Build history of the part. All positions in model axes, mm. Face numbers are marked on the shaded views. A direction names the side the tool comes from. Coordinates: 2 decimals unless noted, no trailing zeros. Write each loop counter-clockwise with the first axis right and the second up, starting at its lowest first coordinate (ties: lowest second). Pieces come first, ordered by that corner, then holes.
from build123d import *

# Parameters (mm, degrees)
BACK_PLATE_PROFILE_W        = 120
BACK_PLATE_PROFILE_H        = 100
BACK_PLATE_120X100X20_DEPTH = 20
TOP_ARM_PROFILE_W           = 120
TOP_ARM_PROFILE_H           = 20
TOP_ARM_80_DEPTH            = 80
SLOT_1_CUT_DEPTH            = 176.499287748
SLOT_2_CUT_DEPTH            = 176.499287748
SLOT_3_CUT_DEPTH            = 176.499287748
ARM_ROOT_FILLET_R10_R       = 10
ARM_CORNER_ROUND_R20_R      = 20
BACK_PLATE_CUT_30_DEPTH     = 176.499287748
BOSS_A_SKETCH_R             = 8
BOSS_A_SKETCH_R_2           = 6
MOUNTING_BOSS_A_DEPTH       = 10
BOSS_B_SKETCH_R             = 8
BOSS_B_SKETCH_R_2           = 6
MOUNTING_BOSS_B_DEPTH       = 10
BOSS_EDGE_FILLET_R2_R       = 2


with BuildPart() as part:
    # Back Plate Profile → Back Plate 120x100x20 (new body)
    with BuildSketch(Plane.XY):
        with Locations((60, 50)):
            Rectangle(BACK_PLATE_PROFILE_W, BACK_PLATE_PROFILE_H)
    extrude(amount=BACK_PLATE_120X100X20_DEPTH)

    # Top Arm Profile → Top Arm 80 (add)
    with BuildSketch(Plane.XY.offset(20)):
        with Locations((60, 90)):
            Rectangle(TOP_ARM_PROFILE_W, TOP_ARM_PROFILE_H)
    extrude(amount=TOP_ARM_80_DEPTH)

    # Slot 1 Sketch → Slot 1 Cut (cut, through all)
    with BuildSketch(Plane.XZ.offset(-80)):
        with BuildLine():
            Line((20, 86), (100, 86))
            ThreePointArc((100, 86), (106, 80), (100, 74))
            Line((100, 74), (20, 74))
            ThreePointArc((20, 74), (14, 80), (20, 86))
        make_face()
    extrude(amount=-SLOT_1_CUT_DEPTH, mode=Mode.SUBTRACT)

    # Slot 2 Sketch → Slot 2 Cut (cut, through all)
    with BuildSketch(Plane.XZ.offset(-80)):
        with BuildLine():
            Line((20, 66), (100, 66))
            ThreePointArc((100, 66), (106, 60), (100, 54))
            Line((100, 54), (20, 54))
            ThreePointArc((20, 54), (14, 60), (20, 66))
        make_face()
    extrude(amount=-SLOT_2_CUT_DEPTH, mode=Mode.SUBTRACT)

    # Slot 3 Sketch → Slot 3 Cut (cut, through all)
    with BuildSketch(Plane.XZ.offset(-80)):
        with BuildLine():
            Line((20, 46.364855501), (100, 46.364855501))
            ThreePointArc((100, 46.364855501), (106.364855501, 40), (100, 33.635144499))
            Line((100, 33.635144499), (20, 33.635144499))
            ThreePointArc((20, 33.635144499), (13.635144499, 40), (20, 46.364855501))
        make_face()
    extrude(amount=-SLOT_3_CUT_DEPTH, mode=Mode.SUBTRACT)

    # Arm Root Fillet R10
    arm_root_fillet_r10_edges = [part.edges().sort_by_distance(p)[0] for p in [
        (60, 80, 20),
    ]]
    fillet(arm_root_fillet_r10_edges, radius=ARM_ROOT_FILLET_R10_R)

    # Arm Corner Round R20
    arm_corner_round_r20_edges = [part.edges().sort_by_distance(p)[0] for p in [
        (0, 90, 100),
        (120, 90, 100),
    ]]
    fillet(arm_corner_round_r20_edges, radius=ARM_CORNER_ROUND_R20_R)

    # Back Plate Cut Sketch → Back Plate Cut 30 (cut, through all)
    with BuildSketch(Plane.XY.offset(20)):
        with BuildLine():
            Line((45, 35), (45, 0))
            Line((45, 0), (75, 0))
            Line((75, 0), (75, 35))
            ThreePointArc((75, 35), (60, 50), (45, 35))
        make_face()
    extrude(amount=-BACK_PLATE_CUT_30_DEPTH, mode=Mode.SUBTRACT)

    # Boss A Sketch → Mounting Boss A (add)
    with BuildSketch(Plane.XY.offset(20)):
        with Locations((30, 30)):
            Circle(BOSS_A_SKETCH_R)
        with Locations((30, 30)):
            Circle(BOSS_A_SKETCH_R_2, mode=Mode.SUBTRACT)
    extrude(amount=MOUNTING_BOSS_A_DEPTH)

    # Boss B Sketch → Mounting Boss B (add)
    with BuildSketch(Plane.XY.offset(20)):
        with Locations((90, 30)):
            Circle(BOSS_B_SKETCH_R)
        with Locations((90, 30)):
            Circle(BOSS_B_SKETCH_R_2, mode=Mode.SUBTRACT)
    extrude(amount=MOUNTING_BOSS_B_DEPTH)

    # Boss Edge Fillet R2
    boss_edge_fillet_r2_edges = [part.edges().sort_by_distance(p)[0] for p in [
        (22, 30, 20),
        (82, 30, 20),
    ]]
    fillet(boss_edge_fillet_r2_edges, radius=BOSS_EDGE_FILLET_R2_R)


solid = part.part
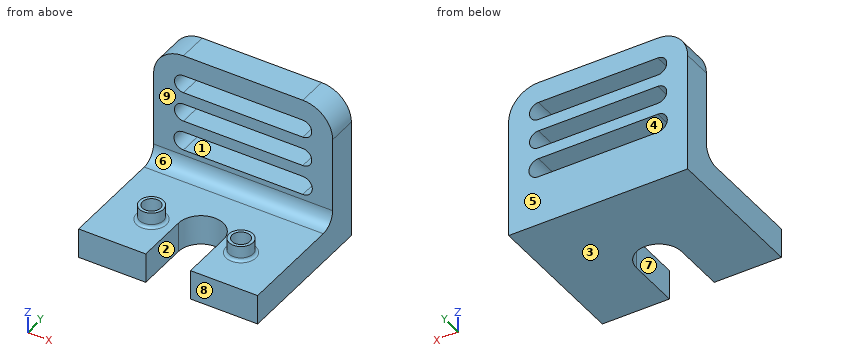
(1) Slice it at B-B, the plane y = 17.5. List the corners of the cut face in (x, z).
(2) Slice it at A-A, the plane x = 30. Give the number of separate pieces and of enclosed holes in the cut face, and give its area (3 significant figures).
(3) Two-plate mould, pull along Z, no slides. Class the marked faces 1, 2, 3 and 4: pulls with the +Z half, pulls with the -Z half, needs draft (parallel to the pull), parting line crosses it, or undercut.
(4) 3-axis set-ups, long thin cutter, end or side, ignore diameter. For the marked faces 5, 6, 7, 8 and 9: which of +Z, -Z, +X, -X, +Y, -Y reach the whole face in a straight line?
(5) Probe L1, parallel to Z at x = 92, y = 93.5; L2, parallel to Y at x = 30, z = 26.25; L3, parallel to Y at x = 90, z = 25.5. List the from-to ranges inside material, lowest first.
(6) Slice it at C-C, the plane z = 60. List the corners of the cut face in (x, y).
(7) Slice it at D-D, the plane z = 12.5. List the corners of the cut face in (x, y).
(8) Flat gauge pins, fed straight in: P1, Ø3.5, axis at x = 92, y = 29, coming from the +Z side; P2, Ø14, axis at x = 90, y = 30, coming from the +Z side; P3, Ø2, axis at x = 106, z = 46.5, coming from the -Y side. Where does each tip first touch, or does it go through?
Results:
1. outline: (0, 0) - (45, 0) - (45, 20) - (0, 20) - close; (75, 0) - (120, 0) - (120, 20) - (75, 20) - close
2. separate pieces: 4
2. enclosed holes: 0
2. area: 2,930 mm2
3. face 1: undercut
3. face 2: needs draft
3. face 3: pulls with the -Z half
3. face 4: undercut
4. face 5: +Z, -Z, +X, -X, +Y
4. face 6: +Z, +X, -X
4. face 7: +Z, -Z, -Y
4. face 8: +Z, -Z, +X, -X, -Y
4. face 9: +Z, +X, -X, -Y
5. L1: z = 0 to 33.64, 46.36 to 54, 66 to 74, 86 to 100
5. L2: y = 22 to 24, 36 to 38, 79.27 to 100
5. L3: y = 22 to 24, 36 to 38, 78.93 to 100
6. outline: (0, 80) - (14, 80) - (14, 100) - (0, 100) - close; (106, 80) - (120, 80) - (120, 100) - (106, 100) - close
7. outline: (0, 0) - (45, 0) - (45, 35) arc R15 cw to (75, 35) - (75, 0) - (120, 0) - (120, 100) - (0, 100) - close
8. P1: stops at z = 20
8. P2: stops at z = 30
8. P3: stops at y = 80
